```python
from build123d import *

# Parameters (mm, degrees)
BOSS_EXTRUDE1_DEPTH = 3


with BuildPart() as part:
    # Sketch1 → Boss-Extrude1 (new body)
    with BuildSketch(Plane.XY):
        with BuildLine():
            Line((0, 0), (30, 0))
            Line((30, 0), (30, 16))
            Line((30, 16), (27, 16))
            Line((27, 16), (27, 8))
            ThreePointArc((27, 8), (23, 4), (19, 8))
            Line((19, 8), (19, 16))
            Line((19, 16), (12, 16))
            Line((12, 16), (12, 8))
            ThreePointArc((12, 8), (8, 4), (4, 8))
            Line((4, 8), (4, 16))
            Line((4, 16), (0, 16))
            Line((0, 16), (0, 0))
        make_face()
    extrude(amount=BOSS_EXTRUDE1_DEPTH)


solid = part.part
```
The listing builds one solid part. Answer for the finished solid, in the listing's coordinates (mm). A direction names the side the tool comes from. Round coordinates to 2 decimals unless told otherwise and drop trailing zeros. Loops run counter-clockwise (first coordinate to the right, second up) from the corner with the lowest first, then second, coordinate; pieces in that order, holes last.
Q1. Section D-D, the plane y = 5.75 is taken. Determine the outline of the cut face in (x, z).
Q2. For a pull along X with two mould halves and no side action, classify faces 3 (the face through (15, 6, 3)), 4 (the face through (8, 4, 1)), 5 (the face through (0, 8, 1)) as released by +X, released by -X, zero draft, split by the parting line, or undercut.
Q3. Which of the six approach directions +Z, -Z, +X, -X, +Y, -Y give full straight-line access (tool end or side, diameter ignored) to faces 1 (the face through (16, 16, 1)), 2 (the face through (27, 12, 1))?
Q4. Find the intervals of material crossed by line 1 (X direction, y = 12.25, z = 2.75); line 2 (X direction, y = 6.5, z = 0.4); line 3 (Y direction, x = 7.25, z = 1.5), in increasing order.
Q5. Section B-B, the plane y = 7.5 is taken. Determine the outline of the cut face in (x, z).
Q6. Section A-A, the plane z = 1.5 is taken. Determine the outline of the cut face in (x, y).
Q7. Section C-C, the plane x = 23 is taken. Determine the outline of the cut face in (y, z), then the cut area to 3 significant figures.
Completed:
1. outline: (0, 0) - (4.69, 0) - (4.69, 3) - (0, 3) - close; (11.31, 0) - (19.69, 0) - (19.69, 3) - (11.31, 3) - close; (26.31, 0) - (30, 0) - (30, 3) - (26.31, 3) - close
2. face 3: zero draft
2. face 4: undercut
2. face 5: released by -X
3. face 1: +Z, -Z, +X, -X, +Y
3. face 2: +Z, -Z, +Y
4. line 1: x = 0 to 4, 12 to 19, 27 to 30
4. line 2: x = 0 to 4.29, 11.71 to 19.29, 26.71 to 30
4. line 3: y = 0 to 4.07
5. outline: (0, 0) - (4.03, 0) - (4.03, 3) - (0, 3) - close; (11.97, 0) - (19.03, 0) - (19.03, 3) - (11.97, 3) - close; (26.97, 0) - (30, 0) - (30, 3) - (26.97, 3) - close
6. outline: (0, 0) - (30, 0) - (30, 16) - (27, 16) - (27, 8) arc R4 cw to (19, 8) - (19, 16) - (12, 16) - (12, 8) arc R4 cw to (4, 8) - (4, 16) - (0, 16) - close
7. outline: (0, 0) - (4, 0) - (4, 3) - (0, 3) - close
7. area: 12.0 mm2
